```python
from build123d import *

# Parameters (mm, degrees)
SKETCH_1_R      = 6
EXTRUDE_1_DEPTH = 59.5
SKETCH_2_W      = 53
SKETCH_2_H      = 14
SKETCH_2_R      = 3
EXTRUDE_2_DEPTH = 4
SKETCH_3_R      = 6.5
EXTRUDE_3_DEPTH = 6.5


with BuildPart() as part:
    # 草图1 → 凸台-拉伸1 (new body)
    with BuildSketch(Plane.XY):
        with Locations(Location((0, 0, 0), (0, 0, 180))):
            Circle(SKETCH_1_R)
    extrude(amount=EXTRUDE_1_DEPTH)

    # 草图2 → 凸台-拉伸2 (add)
    with BuildSketch(Plane(origin=(0, 0, 0), x_dir=(-1, 0, 0), z_dir=(0, 0, -1))):
        Rectangle(SKETCH_2_W, SKETCH_2_H)
        with Locations((-21.5, 0)):
            Circle(SKETCH_2_R, mode=Mode.SUBTRACT)
        with Locations((21.5, 0)):
            Circle(SKETCH_2_R, mode=Mode.SUBTRACT)
    extrude(amount=EXTRUDE_2_DEPTH)

    # 草图3 → 凸台-拉伸3 (add)
    with BuildSketch(Plane.XY):
        with Locations(Location((0, 0, 0), (0, 0, 180))):
            Circle(SKETCH_3_R)
    extrude(amount=EXTRUDE_3_DEPTH)


solid = part.part
```
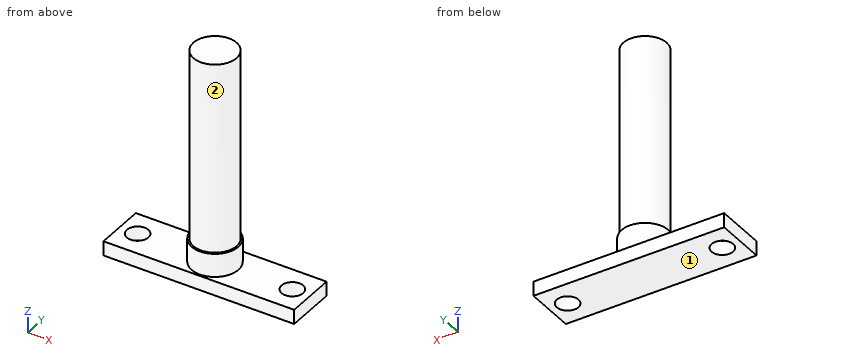
The listing builds one solid part. Answer for the finished solid, in the listing's coordinates (mm). Face numbers are marked on the shaded views. A direction names the side the tool comes from. Give positions to 0.01 mm unless a question says otherwise; leave off trailing zeros. Loops run counter-clockwise (first coordinate to the right, second up) from the corner with the lowest first, then second, coordinate; pieces in that order, holes last. Notation, with made-up numbers: (88, -8) - (96, -8) arc R18 cw to (96, 27) - close; hole circle Ø5 at (56, 59). An arc over 180 degrees is marked (long way). Return JSON: item names as keys, results as strings. Group by question number.
1. Find section A-A (x = 21.5). Write down the section's boundary in (y, z).
2. Find section C-C (y = -3.75). Write down the section's boundary in (x, z).
3. Given pin 1 Ø8 at (x, z) = (17, 7.5) entering from +Y; pin 2 Ø5 at (x, z) = (0.5, 35) entering from +Y; pin 3 Ø1.5 at (y, z) = (-2.5, 6.5) entering from -X; pin 4 Ø4 at (y, z) = (3.5, 28.5) entering from -X, each flat-ended and moving along its own axis, determine where each tip first touches the part or whether it passes through.
4. Straight lines are drawn through the part: line 1 (Y direction, x = -21.5, z = -2.25); line 2 (Z direction, x = 11.5, y = 0.5); line 3 (X direction, y = 5.25, z = 40.5). For each, find the intervals that lie inside material, in ascending order. Write a range as [from, to].
5. Which of the six approach directions +Z, -Z, +X, -X, +Y, -Y give full straight-line access (tool end or side, diameter ignored) to the marked faces 1 and 2?
6. Find section D-D (x = 0). Write down the section's boundary in (y, z), then the cut area to 4 significant figures.
7. Find section B-B (y = 0). Write down the section's boundary in (x, z), then the cut area to 4 significant figures.
Verdict:
{
 "1": {"outline": "(-7, -4) - (-3, -4) - (-3, 0) - (-7, 0) - close; (3, -4) - (7, -4) - (7, 0) - (3, 0) - close"},
 "2": {"outline": "(-26.5, -4) - (26.5, -4) - (26.5, 0) - (5.31, 0) - (5.31, 6.5) - (4.68, 6.5) - (4.68, 59.5) - (-4.68, 59.5) - (-4.68, 6.5) - (-5.31, 6.5) - (-5.31, 0) - (-26.5, 0) - close"},
 "3": {"pin 1": "passes through", "pin 2": "stops at y = 6", "pin 3": "stops at x = -6.26", "pin 4": "stops at x = -5.81"},
 "4": {"line 1": "y = [-7, -3], [3, 7]", "line 2": "z = [-4, 0]", "line 3": "x = [-2.9, 2.9]"},
 "5": {"face 1": "-Z, +X, -X, +Y, -Y", "face 2": "+Z"},
 "6": {"outline": "(-7, -4) - (7, -4) - (7, 0) - (6.5, 0) - (6.5, 6.5) - (6, 6.5) - (6, 59.5) - (-6, 59.5) - (-6, 6.5) - (-6.5, 6.5) - (-6.5, 0) - (-7, 0) - close", "area": "776.5 mm^2"},
 "7": {"outline": "(-26.5, -4) - (-24.5, -4) - (-24.5, 0) - (-26.5, 0) - close; (-18.5, -4) - (18.5, -4) - (18.5, 0) - (6.5, 0) - (6.5, 6.5) - (6, 6.5) - (6, 59.5) - (-6, 59.5) - (-6, 6.5) - (-6.5, 6.5) - (-6.5, 0) - (-18.5, 0) - close; (24.5, -4) - (26.5, -4) - (26.5, 0) - (24.5, 0) - close", "area": "884.5 mm^2"}
}
